For this review, take the finished solid that the model builds, in its own axes (mm). A direction names the side the tool comes from. Coordinates: 2 decimals unless noted, no trailing zeros. Loops run counter-clockwise (first coordinate to the right, second up) from the corner with the lowest first, then second, coordinate; pieces in that order, holes last. Notation, with made-up numbers: (24.5, 20.5) -> (34.5, 20.5) arc R21 ccw to (34.5, 36.5) -> close; hole circle Ø10 at (31.5, 72.5). An arc over 180 degrees is marked (long way). One line per item, written item: value.
from build123d import *

# Parameters (mm, degrees)
SKETCH1_R           = 17.5
BOSS_EXTRUDE1_DEPTH = 105
SKETCH2_R           = 12.5
BOSS_EXTRUDE2_DEPTH = 55
CHAMFER1_SIZE       = 1


with BuildPart() as part:
    # Sketch1 → Boss-Extrude1 (new body)
    with BuildSketch(Plane.XY):
        Circle(SKETCH1_R)
    extrude(amount=BOSS_EXTRUDE1_DEPTH)

    # Sketch2 → Boss-Extrude2 (add)
    with BuildSketch(Plane.XY.offset(105)):
        Circle(SKETCH2_R)
    extrude(amount=BOSS_EXTRUDE2_DEPTH)

    # Chamfer1
    chamfer1_edges = [part.edges().sort_by_distance(p)[0] for p in [
        (-17.5, 0, 0),
        (-12.5, 0, 160),
    ]]
    chamfer(chamfer1_edges, length=CHAMFER1_SIZE)


solid = part.part
1. Insertion check: pin 1 Ø10 at (x, y) = (-11, 11.5) entering from +Z; pin 2 Ø2 at (x, z) = (-4.5, 120) entering from +Y; pin 3 Ø12 at (y, z) = (-11.5, 47) entering from +X; pin 4 Ø2 at (x, z) = (-7.5, 64) entering from +Y. Each pin has a flat end and moves straight along its axis. Give the tip position at first contact, or say it passes through.
Return value:
pin 1: stops at z = 160
pin 2: stops at y = 12
pin 3: stops at x = 16.61
pin 4: stops at y = 16.25
2. Take a section at C-C, the plane z = 36. Give the boundary of the cut face in (x, y).
Return value:
outline: circle Ø35 at (0, 0)
3. To check wall thickness, follow probe 1 along Y at (x, z) = (1, 62.5); probe 2 along Z at (x, y) = (15.5, 1.5); probe 3 along Y at (x, z) = (-8.5, 91). State the ranges of each line that lie inside material, in increasing order. Write a range as from..to.
Return value:
probe 1: y = -17.47..17.47
probe 2: z = 0..105
probe 3: y = -15.3..15.3
4. For faces 1 (the cylindrical face through (-13.887, -10.648, 52.272)), 2 (the flat face through (8, -11, 105)), list the 3-axis set-ups (+Z, -Z, +X, -X, +Y, -Y) from which the entire face can be reached by the end or side of a thin tool; tool diameter is ignored.
Return value:
face 1: +Z, -Z
face 2: +Z
5. Take a section at A-A, the plane x = 0. Give the boundary of the cut face in (y, z), and give its area (3 significant figures).
Return value:
outline: (-17.5, 1) -> (-16.5, 0) -> (16.5, 0) -> (17.5, 1) -> (17.5, 105) -> (12.5, 105) -> (12.5, 159) -> (11.5, 160) -> (-11.5, 160) -> (-12.5, 159) -> (-12.5, 105) -> (-17.5, 105) -> close
area: 5,050 mm2
